Could you check a few things on this model? Use its own coordinates, in mm. Coordinates: 2 decimals unless noted, no trailing zeros. Loops run counter-clockwise (first coordinate to the right, second up) from the corner with the lowest first, then second, coordinate; pieces in that order, holes last. Notation, with made-up numbers: (46, 28) - (54, 28) arc R19 ccw to (54, 33) - close; hole circle Ø6 at (61.25, 68). An arc over 180 degrees is marked (long way). Use CSV: the item, a comma, the result in double quotes.
from build123d import *

# Parameters (mm, degrees)
SKETCH1_W           = 25
SKETCH1_H           = 310
EXTRUDE1_DEPTH      = 6
EXTRUDE3_DEPTH      = 6
SKETCH4_OUTSIDE_W   = 183.172
SKETCH4_OUTSIDE_H   = 378.172
SKETCH4_OUTSIDE_W_2 = 40
SKETCH4_OUTSIDE_H_2 = 128.082699231
CUT_EXTRUDE1_DEPTH  = 22


with BuildPart() as part:
    # Sketch1 → Extrude1 (new, symmetric)
    with BuildSketch(Plane.XY):
        Rectangle(SKETCH1_W, SKETCH1_H)
    extrude(amount=EXTRUDE1_DEPTH, both=True)

    # Sketch3 → Extrude3 (add, symmetric)
    with BuildSketch(Plane.XY):
        Polygon((-12.5, 155), (-72.5, 155), (-102.5, 131), (-102.5, 51), (-12.5, 51), align=None)
        Polygon((-12.5, -51), (-12.5, -155), (-72.5, -155), (-102.5, -131), (-102.5, -51), align=None)
    extrude(amount=EXTRUDE3_DEPTH, both=True)

    # Sketch4 outside → Cut-Extrude1 (cut)
    with BuildSketch(Plane.XY.offset(6)):
        with Locations((-45, 0)):
            Rectangle(SKETCH4_OUTSIDE_W, SKETCH4_OUTSIDE_H)
        with Locations((-82.5, -115.041349616)):
            Rectangle(SKETCH4_OUTSIDE_W_2, SKETCH4_OUTSIDE_H_2, mode=Mode.SUBTRACT)
    extrude(amount=-CUT_EXTRUDE1_DEPTH, mode=Mode.SUBTRACT)


solid = part.part
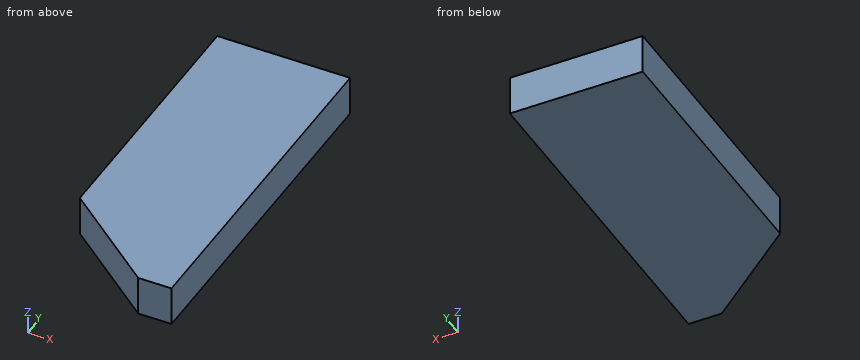
(1) Suppose I cut it at C-C (y = -133). Write out the boundary of the cut face in (x, z).
Computed:
outline,"(-100, -6) - (-62.5, -6) - (-62.5, 6) - (-100, 6) - close"
(2) Suppose I cut it at A-A (z = -0.5). Write out the boundary of the cut face in (x, y), plus the area to 3 significant figures.
Computed:
outline,"(-102.5, -131) - (-72.5, -155) - (-62.5, -155) - (-62.5, -51) - (-102.5, -51) - close"
area,"3,800 mm²"
(3) Suppose I cut it at B-B (x = -80.5). Write out the boundary of the cut face in (y, z).
Computed:
outline,"(-148.6, -6) - (-51, -6) - (-51, 6) - (-148.6, 6) - close"
(4) Please list where these lines run through material, in increasing order: line 1 (Y direction, x = -91.5, z = -5); line 2 (Y direction, x = -95.5, z = 3.5).
Computed:
line 1,"y = -139.8 to -51"
line 2,"y = -136.6 to -51"
